from build123d import *

# Parameters (mm, degrees)
SKETCH_1_W          = 360
SKETCH_1_H          = 220
EXTRUDE_1_DEPTH     = 30
SKETCH_2_R          = 40
CUT_EXTRUDE_1_DEPTH = 214.072757527
SKETCH_3_R          = 45
CUT_EXTRUDE_2_DEPTH = 20


with BuildPart() as part:
    # 草图1 → 凸台-拉伸1 (new body)
    with BuildSketch(Plane(origin=(0, 0, 0), x_dir=(1, 0, 0), z_dir=(0, 1, 0))):
        Rectangle(SKETCH_1_W, SKETCH_1_H)
    extrude(amount=EXTRUDE_1_DEPTH)

    # 草图2 → 切除-拉伸1 (cut, through all)
    with BuildSketch(Plane(origin=(0, 30, 0), x_dir=(1, 0, 0), z_dir=(0, 1, 0))):
        with Locations(Location((0, -45, 0), (0, 0, 270))):
            Circle(SKETCH_2_R)
    extrude(amount=-CUT_EXTRUDE_1_DEPTH, mode=Mode.SUBTRACT)

    # 草图3 → 切除-拉伸2 (cut)
    with BuildSketch(Plane.XZ.offset(-30)):
        with Locations(Location((0, 45, 0), (0, 0, 270))):
            Circle(SKETCH_3_R)
    extrude(amount=CUT_EXTRUDE_2_DEPTH, mode=Mode.SUBTRACT)


solid = part.part
The model under review builds one solid part; all positions refer to its coordinate system, in mm. A direction names the side the tool comes from. Round coordinates to 2 decimals unless told otherwise and drop trailing zeros. Write each loop counter-clockwise with the first axis right and the second up, starting at its lowest first coordinate (ties: lowest second). Pieces come first, ordered by that corner, then holes. Notation, with made-up numbers: M -39.5,15.5 L -19.5,15.5 A6 ccw -19.5,21.5 Z; hole C 0.5,53 d7. An arc over 180 degrees is marked long. Answer as CSV lines item,"result". Start each with the question number.
Q1. The part is to be moulded in two halves that separate along Z. For faces 3 (the face through (1.76, 5.07, 5.04)), 4 (the face through (-3, 30, -2)), 5 (the face through (-3, 15, -110)), 6 (the face through (1.979, 20.14, 89.956)), say which applies: +Z half, -Z half, draft (parallel to the pull), parting line (faces both ways), or undercut.
Q2. Consider section A-A, the plane z = 45. Give the boundary of the cut face in (x, y).
Q3. Wall thickness on line 1 along X through (y, z) = (6.25, 45); line 2 along Z through (x, y) = (6.5, 24.5); line 3 along Z through (x, y) = (-2.5, 10.5): over which ranges is each line inside the solid? List them lowest first.
Q4. Tool access review of faces 1 (the face through (180, 15, 2)), 2 (the face through (-26.5, 10, 75.2)): name each direction out of +Z, -Z, +X, -X, +Y, -Y from which nothing blocks a thin tool from reaching the whole face with its end or side.
Q5. Consider section B-B, the plane x = 0. Give the boundary of the cut face in (y, z), then the cut area to 3 significant figures.
Q6. Consider section C-C, the plane y = 5.75. Give the boundary of the cut face in (x, z).
Result set:
1,face 3,"undercut"
1,face 4,"draft"
1,face 5,"-Z half"
1,face 6,"undercut"
2,outline,"M -180,0 L -40,0 L -40,10 L -45,10 L -45,30 L -180,30 Z; M 40,0 L 180,0 L 180,30 L 45,30 L 45,10 L 40,10 Z"
3,line 1,"x = -180 to -40, 40 to 180"
3,line 2,"z = -110 to 0.47, 89.53 to 110"
3,line 3,"z = -110 to 0.07, 89.93 to 110"
4,face 1,"+Z, -Z, +X, +Y, -Y"
4,face 2,"+Y"
5,outline,"M 0,-110 L 30,-110 L 30,0 L 10,0 L 10,5 L 0,5 Z; M 0,85 L 10,85 L 10,90 L 30,90 L 30,110 L 0,110 Z"
5,area,"4,000 mm²"
6,outline,"M -180,-110 L 180,-110 L 180,110 L -180,110 Z; hole C 0,45 d80"
